from build123d import *

# Parameters (mm, degrees)
BASE_PLATE_DEPTH            = 15
BASE_BORE_SKETCH_R          = 15
BASE_BORE_DEPTH             = 15
LOOP_START                  = -10
LOOP_RING_DEPTH             = 50
BRACE_ANGLE_CUT_DEPTH       = 223.261107709
X_BRACE_WEB_DEPTH           = 10
BRACE_TRIM_CUT_SKETCH_R     = 15
BRACE_TRIM_CUT_DEPTH        = 10
INNER_PLATE_DEPTH           = 10
INNER_PLATE_EXTENSION_DEPTH = 10


with BuildPart() as part:
    # Base Plate Sketch → Base Plate (new body)
    with BuildSketch(Plane(origin=(0, 0, 0), x_dir=(1, 0, 0), z_dir=(0, 1, 0))):
        with BuildLine():
            Line((0, 50), (100, 50))
            ThreePointArc((100, 50), (150, 0), (100, -50))
            Line((100, -50), (0, -50))
            ThreePointArc((0, -50), (-50, 0), (0, 50))
        make_face()
    extrude(amount=BASE_PLATE_DEPTH)

    # Base Bore Sketch → Base Bore (cut)
    with BuildSketch(Plane(origin=(0, 15, 0), x_dir=(1, 0, 0), z_dir=(0, 1, 0))):
        with Locations(Location((100, 0, 0), (0, 0, 270))):
            Circle(BASE_BORE_SKETCH_R)
        with Locations(Location((0, 0, 0), (0, 0, 270))):
            Circle(BASE_BORE_SKETCH_R)
    extrude(amount=-BASE_BORE_DEPTH, mode=Mode.SUBTRACT)



with BuildPart() as body_2:
    # Loop Ring Sketch → Loop Ring (new body)
    with BuildSketch(Plane(origin=(0, 90, 0), x_dir=(1, 0, 0), z_dir=(0, 1, 0)).offset(LOOP_START)):
        with BuildLine():
            Line((0, -50), (100, -50))
            ThreePointArc((100, -50), (150, 0), (100, 50))
            Line((100, 50), (0, 50))
            ThreePointArc((0, 50), (-50, 0), (0, -50))
        make_face()
        with BuildLine():
            Line((0, 40), (100, 40))
            ThreePointArc((100, 40), (140, 0), (100, -40))
            Line((100, -40), (0, -40))
            ThreePointArc((0, -40), (-40, 0), (0, 40))
        make_face(mode=Mode.SUBTRACT)
    extrude(amount=LOOP_RING_DEPTH)

    # Brace Angle Cut Sketch → Brace Angle Cut (cut, through all)
    with BuildSketch(Plane.XY.offset(50)):
        Polygon((150, 90), (150, 130), (-50, 130), (-50, 125.265396142), align=None)
    extrude(amount=-BRACE_ANGLE_CUT_DEPTH, mode=Mode.SUBTRACT)

    # X-Brace Sketch → X-Brace Web (add)
    with BuildSketch(Plane(origin=(0, 90, 0), x_dir=(1, 0, 0), z_dir=(0, 1, 0))):
        with BuildLine():
            Line((0, 25), (75, 25))
            Line((75, 25), (75, 40))
            Line((75, 40), (100, 40))
            Line((100, 40), (100, 25))
            ThreePointArc((100, 25), (125, 0), (100, -25))
            Line((100, -25), (25, -25))
            Line((25, -25), (25, -40))
            Line((25, -40), (0, -40))
            Line((0, -40), (0, -25))
            ThreePointArc((0, -25), (-25, 0), (0, 25))
        make_face()
    extrude(amount=-X_BRACE_WEB_DEPTH)

    # Brace Trim Cut Sketch → Brace Trim Cut (cut)
    with BuildSketch(Plane(origin=(0, 90, 0), x_dir=(1, 0, 0), z_dir=(0, 1, 0))):
        with Locations(Location((100, 0, 0), (0, 0, 270))):
            Circle(BRACE_TRIM_CUT_SKETCH_R)
        with Locations(Location((0, 0, 0), (0, 0, 270))):
            Circle(BRACE_TRIM_CUT_SKETCH_R)
    extrude(amount=-BRACE_TRIM_CUT_DEPTH, mode=Mode.SUBTRACT)


with BuildPart() as part_1:
    add(part.part)

    add(body_2.part)  # Inner Plate merges body 2
    # Inner Plate Sketch → Inner Plate (add)
    with BuildSketch(Plane.XY.offset(50)):
        Polygon((0, 80), (75, 15), (100, 15), (25, 80), align=None)
    extrude(amount=-INNER_PLATE_DEPTH)

    # Inner Plate Extension Sketch → Inner Plate Extension (add)
    with BuildSketch(Plane(origin=(0, 0, -50), x_dir=(-1, 0, 0), z_dir=(0, 0, -1))):
        Polygon((-100, 80), (-25, 15), (0, 15), (-75, 80), align=None)
    extrude(amount=-INNER_PLATE_EXTENSION_DEPTH)


solid = part_1.part
Can you work these out from the model? Positions are in its coordinate system, mm. A direction names the side the tool comes from. Round coordinates to 2 decimals unless told otherwise and drop trailing zeros. Write each loop counter-clockwise with the first axis right and the second up, starting at its lowest first coordinate (ties: lowest second). Pieces come first, ordered by that corner, then holes. Notation, with made-up numbers: M 83.5,-5 L 98.5,-5 A32 cw 98.5,24 Z; hole C 44,49.25 d11. An arc over 180 degrees is marked long. Use a Markdown table: item, result.
Item 1: I want a section at A-A (x = 121). List the corners of the cut face in (y, z) for me.
Found:
| item | result |
|---|---|
| outline | M 0,-45.38 L 15,-45.38 L 15,45.38 L 0,45.38 Z; M 80,-45.38 L 95.11,-45.38 L 95.11,-34.04 L 80,-34.04 Z; M 80,-13.56 L 90,-13.56 L 90,13.56 L 80,13.56 Z; M 80,34.04 L 95.11,34.04 L 95.11,45.38 L 80,45.38 Z |
Item 2: I want a section at C-C (x = -9). List the corners of the cut face in (y, z) for me.
Found:
| item | result |
|---|---|
| outline | M 0,-49.18 L 15,-49.18 L 15,-12 L 0,-12 Z; M 0,12 L 15,12 L 15,49.18 L 0,49.18 Z; M 80,-49.18 L 118.04,-49.18 L 118.04,-38.97 L 80,-38.97 Z; M 80,-23.32 L 90,-23.32 L 90,-12 L 80,-12 Z; M 80,12 L 90,12 L 90,23.32 L 80,23.32 Z; M 80,38.97 L 118.04,38.97 L 118.04,49.18 L 80,49.18 Z |
Item 3: I want a section at D-D (z = 7). State how many separate pieces and enclosed holes the cut face has, and give its area (3 significant figures).
Found:
| item | result |
|---|---|
| separate pieces | 8 |
| enclosed holes | 0 |
| area | 3,700 mm2 |
Item 4: We'd pull the mould along Y, two halves only. Please class faces 1 (the face through (63, 85, 25)), 2 (the face through (-1, 80, -41)), 3 (the face through (51, 90, -1)), 4 (the face through (51, 15, -1)): released by +Y, released by -Y, zero draft, split by the parting line, or undercut.
Found:
| item | result |
|---|---|
| face 1 | zero draft |
| face 2 | undercut |
| face 3 | released by +Y |
| face 4 | undercut |
Item 5: Which directions (+Z, -Z, +X, -X, +Y, -Y) give clear straight access to the entire face, cutting with the end or side of a thin tool? Please do faces 5 (the face through (50, 50, -40)), 6 (the face through (62, 59, -50)), 7 (the face through (124.994, 85.07, -0.55)).
Found:
| item | result |
|---|---|
| face 5 | +X, -X |
| face 6 | -Z, +X, -X, +Y, -Y |
| face 7 | +Y |
Item 6: For pin 1 Ø8 at (y, z) = (84.5, 33) entering from -X; pin 2 Ø4 at (x, z) = (15.5, -13.5) entering from +Y; pin 3 Ø3 at (x, z) = (0, -37) entering from +Y, each with a flat end and sliding along its axis, tell me the tip position at first contact or that it passes through.
Found:
| item | result |
|---|---|
| pin 1 | stops at x = -40.73 |
| pin 2 | stops at y = 90 |
| pin 3 | stops at y = 15 |
Item 7: If I drill on line 1 along X through (y, z) = (84, 0); line 2 along X through (y, z) = (8.5, 0); line 3 along Z through (x, y) = (40.5, 83), over which ranges is the centre line in solid material (lowest first)? Write a range as [from, to].
Found:
| item | result |
|---|---|
| line 1 | x = [-50, -40], [-25, -15], [15, 85], [115, 125], [140, 150] |
| line 2 | x = [-50, -15], [15, 85], [115, 150] |
| line 3 | z = [-50, -40], [-25, 25], [40, 50] |
Item 8: I want a section at B-B (z = -28.5). List the corners of the cut face in (x, y) for me, and give its area (3 significant figures).
Found:
| item | result |
|---|---|
| outline | M -41.08,0 L 141.08,0 L 141.08,15 L -41.08,15 Z; M -41.08,80 L -28.07,80 L -28.07,121.4 L -41.08,123.69 Z; M 75,80 L 100,80 L 100,90 L 75,90 Z; M 128.07,80 L 141.08,80 L 141.08,91.57 L 128.07,93.87 Z |
| area | 3,700 mm2 |
